Could you check a few things on this model? Use its own coordinates, in mm. Give positions to 0.01 mm unless a question says otherwise; leave off trailing zeros. Loops run counter-clockwise (first coordinate to the right, second up) from the corner with the lowest first, then second, coordinate; pieces in that order, holes last. Notation, with made-up numbers: (80.25, 70.5) - (113.25, 70.5) arc R14 ccw to (113.25, 94.5) - close; hole circle Ø5 at (34.25, 18.5). An arc over 180 degrees is marked (long way). One line per item, written item: value. Start each with the question number.
Q1. I want a section at B-B (z = 94). Please give me the cut outline in (x, y), then the cut area to 3 significant figures.
Q2. If I drill on line 1 (X direction, y = 22.6, z = 738); line 2 (Y direction, x = -22.5, z = 224.5), over which ranges is the centre line in solid material (lowest first)? Write a range as from..to.
Q3. I want a section at A-A (x = -25.25). Please give me the cut outline in (y, z), then the cut area to 3 significant figures.
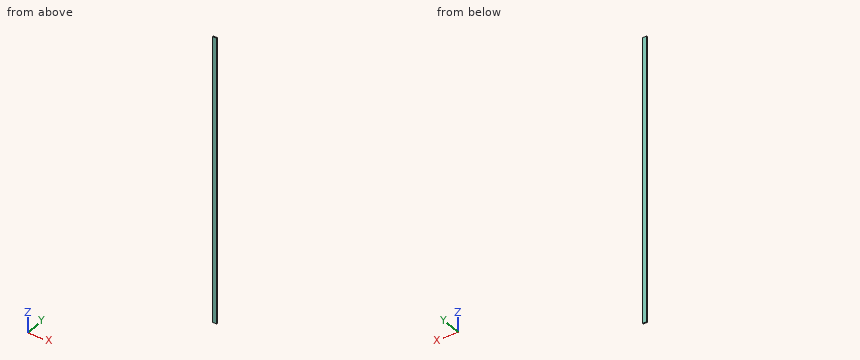
```python
from build123d import *

# Parameters (mm, degrees)
SKETCH1_W           = 12
SKETCH1_H           = 3
BOSS_EXTRUDE1_DEPTH = 840
SKETCH2_W           = 10
SKETCH2_H           = 1
CUT_EXTRUDE1_DEPTH  = 841.951655259


with BuildPart() as part:
    # Sketch1 → Boss-Extrude1 (new body)
    with BuildSketch(Plane.XY):
        with Locations((-25.901003365, 22.624934563)):
            Rectangle(SKETCH1_W, SKETCH1_H)
    extrude(amount=BOSS_EXTRUDE1_DEPTH)

    # Sketch2 → Cut-Extrude1 (cut, through all)
    with BuildSketch(Plane.XY.offset(840)):
        with Locations((-25.901003365, 22.624934563)):
            Rectangle(SKETCH2_W, SKETCH2_H)
    extrude(amount=-CUT_EXTRUDE1_DEPTH, mode=Mode.SUBTRACT)


solid = part.part
```
Worked answers:
1. outline: (-31.9, 21.12) - (-19.9, 21.12) - (-19.9, 24.12) - (-31.9, 24.12) - close; hole (-30.9, 22.12) - (-20.9, 22.12) - (-20.9, 23.12) - (-30.9, 23.12) - close
1. area: 26.0 mm²
2. line 1: x = -31.9..-30.9, -20.9..-19.9
2. line 2: y = 21.12..22.12, 23.12..24.12
3. outline: (21.12, 0) - (22.12, 0) - (22.12, 840) - (21.12, 840) - close; (23.12, 0) - (24.12, 0) - (24.12, 840) - (23.12, 840) - close
3. area: 1,680 mm²
